Build history of the part. All positions in model axes, mm. Face numbers are marked on the shaded views. A direction names the side the tool comes from. Coordinates: 2 decimals unless noted, no trailing zeros. Loops run counter-clockwise (first coordinate to the right, second up) from the corner with the lowest first, then second, coordinate; pieces in that order, holes last.
Item 1: Cut at C-C (x = -20). List the corners of the cut face in (y, z).
Item 2: Cut at D-D (y = 0). List the corners of the cut face in (x, z), and give its area (3 significant figures).
Item 3: 3-axis set-ups, long thin cutter, end or side, ignore diameter. For the marked faces 4 and 5: which of +Z, -Z, +X, -X, +Y, -Y reach the whole face in a straight line?
Item 4: Mould opens along Y. For the marked faces 1, 2 and 3 say: released by +Y, released by -Y, zero draft, split by the parting line, or undercut.
Item 5: Drill centre lines: line 1 along Y through (x, z) = (-6, 35); line 2 along X through (y, z) = (-9.5, 41); line 3 along Y through (x, z) = (23, 20). Where is each one in solid material? Low to high.
Item 6: Cut at A-A (y = 27). List the corners of the cut face in (x, z).
Item 7: Cut at B-B (z = 20). List the corners of the cut face in (x, y).
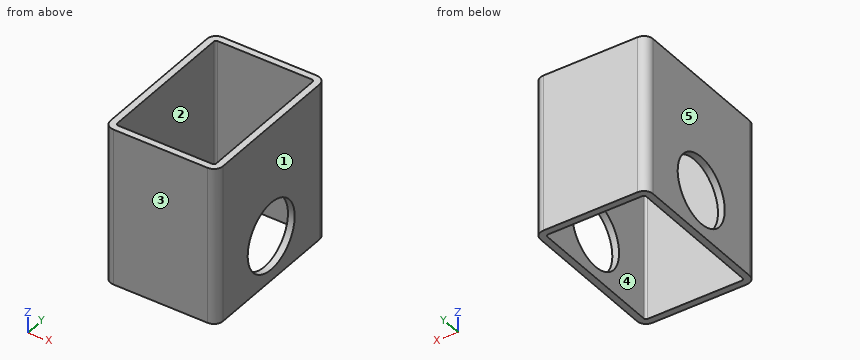
from build123d import *

# Parameters (mm, degrees)
EXTRUDE_THIN1_DEPTH = 70
SKETCH2_R           = 15.1
CUT_EXTRUDE1_DEPTH  = 93.870878105


with BuildPart() as part:
    # Sketch1 → Extrude-Thin1 (new body)
    with BuildSketch(Plane.XY):
        with BuildLine():
            Line((-25, 31), (-25, -31))
            ThreePointArc((-25, -31), (-23.828427125, -33.828427125), (-21, -35))
            Line((-21, -35), (21, -35))
            ThreePointArc((21, -35), (23.828427125, -33.828427125), (25, -31))
            Line((25, -31), (25, 31))
            ThreePointArc((25, 31), (23.828427125, 33.828427125), (21, 35))
            Line((21, 35), (-21, 35))
            ThreePointArc((-21, 35), (-23.828427125, 33.828427125), (-25, 31))
        make_face()
        with BuildLine():
            Line((-22, 31), (-22, -31))
            ThreePointArc((-22, -31), (-21.707106781, -31.707106781), (-21, -32))
            Line((-21, -32), (21, -32))
            ThreePointArc((21, -32), (21.707106781, -31.707106781), (22, -31))
            Line((22, -31), (22, 31))
            ThreePointArc((22, 31), (21.707106781, 31.707106781), (21, 32))
            Line((21, 32), (-21, 32))
            ThreePointArc((-21, 32), (-21.707106781, 31.707106781), (-22, 31))
        make_face(mode=Mode.SUBTRACT)
    extrude(amount=EXTRUDE_THIN1_DEPTH)

    # Sketch2 → Cut-Extrude1 (cut, through all)
    with BuildSketch(Plane(origin=(25, 0, 0), x_dir=(0, 0, -1), z_dir=(1, 0, 0))):
        with Locations((-20, 0)):
            Circle(SKETCH2_R)
    extrude(amount=-CUT_EXTRUDE1_DEPTH, mode=Mode.SUBTRACT)


solid = part.part
Filled sheet:
1. outline: (-35, 0) - (-32, 0) - (-32, 70) - (-35, 70) - close; (32, 0) - (35, 0) - (35, 70) - (32, 70) - close
2. outline: (-25, 0) - (-22, 0) - (-22, 4.9) - (-25, 4.9) - close; (-25, 35.1) - (-22, 35.1) - (-22, 70) - (-25, 70) - close; (22, 0) - (25, 0) - (25, 4.9) - (22, 4.9) - close; (22, 35.1) - (25, 35.1) - (25, 70) - (22, 70) - close
2. area: 239 mm2
3. face 4: +Z, -Z
3. face 5: +Z, -Z, -X, +Y, -Y
4. face 1: zero draft
4. face 2: undercut
4. face 3: released by -Y
5. line 1: y = -35 to -32, 32 to 35
5. line 2: x = -25 to -22, 22 to 25
5. line 3: y = -34.46 to -15.1, 15.1 to 34.46
6. outline: (-25, 0) - (-22, 0) - (-22, 70) - (-25, 70) - close; (22, 0) - (25, 0) - (25, 70) - (22, 70) - close
7. outline: (-25, -31) arc R4 ccw to (-21, -35) - (21, -35) arc R4 ccw to (25, -31) - (25, -15.1) - (22, -15.1) - (22, -31) arc R1 cw to (21, -32) - (-21, -32) arc R1 cw to (-22, -31) - (-22, -15.1) - (-25, -15.1) - close; (-25, 15.1) - (-22, 15.1) - (-22, 31) arc R1 cw to (-21, 32) - (21, 32) arc R1 cw to (22, 31) - (22, 15.1) - (25, 15.1) - (25, 31) arc R4 ccw to (21, 35) - (-21, 35) arc R4 ccw to (-25, 31) - close
